from build123d import *

# Parameters (mm, degrees)
SKETCH_2_R      = 1.8
EXTRUDE_1_DEPTH = 7
SKETCH_3_R      = 0.75
EXTRUDE_2_DEPTH = 8.9
CHAMFER_1_SIZE  = 0.5
CHAMFER_2_SIZE  = 0.5
SKETCH_4_R      = 1.4
EXTRUDE_3_DEPTH = 1.9
CHAMFER_3_SIZE  = 0.5


with BuildPart() as part:
    # 草图2 → 拉伸1 (new body)
    with BuildSketch(Plane.XY):
        Circle(SKETCH_2_R)
    extrude(amount=EXTRUDE_1_DEPTH)

    # 草图3 → 拉伸2 (add)
    with BuildSketch(Plane.XY.offset(7)):
        Circle(SKETCH_3_R)
    extrude(amount=EXTRUDE_2_DEPTH)

    # 倒角1
    chamfer_1_edges = [part.edges().sort_by_distance(p)[0] for p in [
        (-1.8, 0, 0),
    ]]
    chamfer(chamfer_1_edges, length=CHAMFER_1_SIZE)

    # 倒角2
    chamfer_2_edges = [part.edges().sort_by_distance(p)[0] for p in [
        (-1.8, 0, 7),
    ]]
    chamfer(chamfer_2_edges, length=CHAMFER_2_SIZE)

    # 草图4 → 拉伸3 (add)
    with BuildSketch(Plane(origin=(0, 0, 0), x_dir=(-1, 0, 0), z_dir=(0, 0, -1))):
        with Locations(Location((0, 0, 0), (0, 0, 180))):
            Circle(SKETCH_4_R)
    extrude(amount=EXTRUDE_3_DEPTH)

    # 倒角3
    chamfer_3_edges = [part.edges().sort_by_distance(p)[0] for p in [
        (-1.4, 0, -1.9),
    ]]
    chamfer(chamfer_3_edges, length=CHAMFER_3_SIZE)


solid = part.part
Input: part model. Units: mm. Frame: model coordinates. A direction names the side the tool comes from. Round coordinates to 2 decimals unless told otherwise and drop trailing zeros. Order: outer loops, then holes, each group sorted by start corner. A loop starts at its lowest first (then second) coordinate and runs counter-clockwise, first axis right, second up. Notation, with made-up numbers: (15, 58.25) - (31, 58.25) arc R7 cw to (31, 64.25) - close; hole circle Ø11 at (5, -38.75). An arc over 180 degrees is marked (long way). Answer as a JSON object with one key per item and string values. Group by question number.
(1) Reachability of faces 1 (the face through (0, 0, -1.9)), 2 (the face through (1, 0, 7)), 3 (the face through (-1.4, -0.06, -0.69)) from +Z, -Z, +X, -X, +Y, -Y: full face, straight path, thin tool, end or side. Return the list, or none.
(2) Cut plane D-D (z = 13.75). Return loops of the section in (x, y), then the cut area to 3 significant figures.
(3) Pin query (flat end, axial travel): P1, Ø2, axis at x = 0, z = 14, coming from the -Y side; P2, Ø1, axis at y = 0.5, z = 10, coming from the -X side. Return the tip coordinate at first contact, or that it passes through.
(4) Cut plane A-A (x = 0). Return loops of the section in (y, z).
(5) Cut plane C-C (z = 4). Return loops of the section in (x, y), then the cut area to 3 significant figures.
(6) Material intervals for probe 1 along Z at (x, y) = (0.05, 1); probe 2 along Y at (x, z) = (-0.4, 6.75); probe 3 along Z at (x, y) = (0.4, 1.6), sorted ascending. Write a range as from..to.
Here are the results:
{
 "1": {"face 1": "-Z, +X, -X, +Y, -Y", "face 2": "+Z", "face 3": "-Z"},
 "2": {"outline": "circle Ø1.5 at (0, 0)", "area": "1.77 mm^2"},
 "3": {"P1": "stops at y = -0.75", "P2": "stops at x = -0.75"},
 "4": {"outline": "(-1.8, 0.5) - (-1.3, 0) - (-1.4, 0) - (-1.4, -1.4) - (-0.9, -1.9) - (0.9, -1.9) - (1.4, -1.4) - (1.4, 0) - (1.3, 0) - (1.8, 0.5) - (1.8, 6.5) - (1.3, 7) - (0.75, 7) - (0.75, 15.9) - (-0.75, 15.9) - (-0.75, 7) - (-1.3, 7) - (-1.8, 6.5) - close"},
 "5": {"outline": "circle Ø3.6 at (0, 0)", "area": "10.2 mm^2"},
 "6": {"probe 1": "z = -1.8..7", "probe 2": "y = -1.5..1.5", "probe 3": "z = 0.35..6.65"}
}
